The model under review builds one solid part; all positions refer to its coordinate system, in mm. Face numbers are marked on the shaded views. Give positions to 0.01 mm unless a question says otherwise; leave off trailing zeros. Write each loop counter-clockwise with the first axis right and the second up, starting at its lowest first coordinate (ties: lowest second). Pieces come first, ordered by that corner, then holes. Notation, with made-up numbers: (68.5, -38) -> (99.5, -38) arc R17 ccw to (99.5, -32) -> close; hole circle Ø7 at (44.25, -37.5). An arc over 180 degrees is marked (long way). Use CSV: the item, a comma, the result in double quotes.
```python
from build123d import *

# Parameters (mm, degrees)
SKETCH1_R           = 8
BOSS_EXTRUDE1_DEPTH = 8


with BuildPart() as part:
    # Sketch1 → Boss-Extrude1 (new body)
    with BuildSketch(Plane.XY):
        with BuildLine():
            Line((-20, 0), (-20, -25))
            Line((-20, -25), (20, -25))
            Line((20, -25), (20, 0))
            ThreePointArc((20, 0), (0, 20), (-20, 0))
        make_face()
        Circle(SKETCH1_R, mode=Mode.SUBTRACT)
    extrude(amount=BOSS_EXTRUDE1_DEPTH)


solid = part.part
```
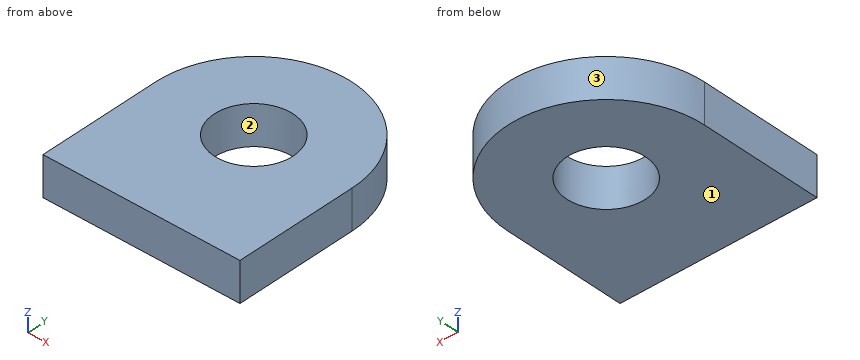
Q1. To check wall thickness, follow probe 1 along Y at (x, z) = (0, 6.25); probe 2 along X at (y, z) = (0.5, 5); probe 3 along X at (y, z) = (5, 1) (3 decimals). State the ranges of each line that lie inside material, in increasing order.
Derived:
probe 1,"y = -25 to -8, 8 to 20"
probe 2,"x = -19.99 to -7.98, 7.98 to 19.99"
probe 3,"x = -19.365 to -6.245, 6.245 to 19.365"
Q2. Consider section B-B (y = 7.5). Write out the cut boundary in (x, z).
Derived:
outline,"(-18.54, 0) -> (-2.78, 0) -> (-2.78, 8) -> (-18.54, 8) -> close; (2.78, 0) -> (18.54, 0) -> (18.54, 8) -> (2.78, 8) -> close"
Q3. Consider section A-A (x = 0). Write out the cut boundary in (y, z), then the cut area to 3 significant figures.
Derived:
outline,"(-25, 0) -> (-8, 0) -> (-8, 8) -> (-25, 8) -> close; (8, 0) -> (20, 0) -> (20, 8) -> (8, 8) -> close"
area,"232 mm2"
Q4. Consider section D-D (x = 10). Write out the cut boundary in (y, z).
Derived:
outline,"(-25, 0) -> (17.32, 0) -> (17.32, 8) -> (-25, 8) -> close"
Q5. Insertion check: pin 1 (3 mm diameter, centred on x = 5.5, z = 4, fed in from +Y); pin 2 (3 mm diameter, centred on x = -10, z = 2, fed in from +Y). Each pin has a flat end and moves straight along its axis. Give the tip position at first contact, or say it passes through.
Derived:
pin 1,"stops at y = 19.6"
pin 2,"stops at y = 18.1"
Q6. Consider section C-C (z = 5.25). Write out the cut boundary in (x, y), then the cut area to 3 significant figures.
Derived:
outline,"(-20, -25) -> (20, -25) -> (20, 0) arc R20 ccw to (-20, 0) -> close; hole circle Ø16 at (0, 0)"
area,"1,430 mm2"
Q7. The part is to be moulded in two halves that separate along X. For the marked faces 1, 2 and 3, say which applies: pulls with the +X half, pulls with the -X half, needs draft (parallel to the pull), parting line crosses it, or undercut.
Derived:
face 1,"needs draft"
face 2,"undercut"
face 3,"parting line crosses it"
